```python
from build123d import *

# Parameters (mm, degrees)
EXTRUDE_THIN1_DEPTH = 372
SKETCH2_R           = 4.5
CUT_EXTRUDE1_DEPTH  = 447.144595395
LPATTERN1_COUNT     = 2
LPATTERN1_PITCH     = 320


with BuildPart() as part:
    # Sketch1 → Extrude-Thin1 (new body)
    with BuildSketch(Plane.XY):
        with BuildLine():
            Line((50, 206), (10, 206))
            ThreePointArc((10, 206), (2.928932188, 203.071067812), (0, 196))
            Line((0, 196), (0, 10))
            ThreePointArc((0, 10), (2.928932188, 2.928932188), (10, 0))
            Line((10, 0), (135, 0))
            Line((135, 0), (135, 5))
            Line((135, 5), (10, 5))
            ThreePointArc((10, 5), (6.464466094, 6.464466094), (5, 10))
            Line((5, 10), (5, 196))
            ThreePointArc((5, 196), (6.464466094, 199.535533906), (10, 201))
            Line((10, 201), (50, 201))
            Line((50, 201), (50, 206))
        make_face()
    extrude(amount=EXTRUDE_THIN1_DEPTH)

    # Sketch2 → Cut-Extrude1 (cut, through all)
    with BuildSketch(Plane(origin=(0, 206, 0), x_dir=(1, 0, 0), z_dir=(0, 1, 0))):
        with Locations(Location((27.5, -346, 0), (0, 0, 270))):
            Circle(SKETCH2_R)
    cut_extrude1 = extrude(amount=-CUT_EXTRUDE1_DEPTH, mode=Mode.SUBTRACT)

    # LPattern1: Cut-Extrude1 ×2
    with Locations(*[(0, 0, -i * LPATTERN1_PITCH) for i in range(1, LPATTERN1_COUNT)]):
        add(cut_extrude1, mode=Mode.SUBTRACT)


solid = part.part
```
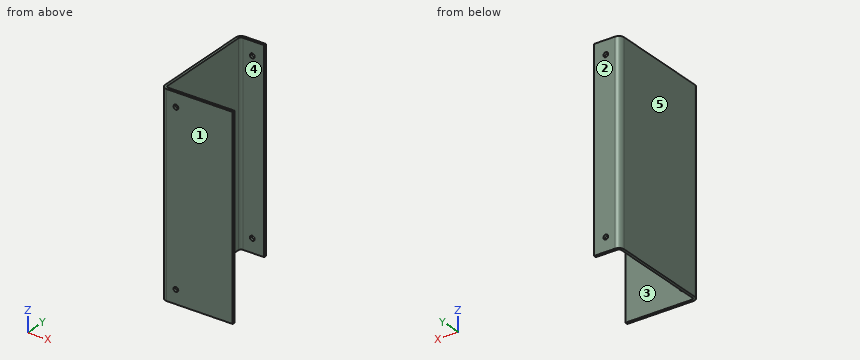
Geometry: final body of the model. Coordinates: model frame, mm. Face numbers are marked on the shaded views. A direction names the side the tool comes from. Coordinates: 2 decimals unless noted, no trailing zeros. Order: outer loops, then holes, each group sorted by start corner. A loop starts at its lowest first (then second) coordinate and runs counter-clockwise, first axis right, second up. Notation, with made-up numbers: (14, 65) - (47, 65) arc R21 cw to (47, 86) - close; hole circle Ø11 at (32.5, 53.5). An arc over 180 degrees is marked (long way). Return JSON: item names as keys, results as strings. Group by question number.
1. Cut plane A-A (x = 27.5). Output: boundary loops of the cut face in (y, z).
2. Material intervals for line 1 along Z through (x, y) = (27, 2); line 2 along Y through (x, z) = (45, 217.5); line 3 along X through (y, z) = (181.5, 139), sorted ascending. Write a range as [from, to].
3. Pull-direction query (Y, two-part tool) for the marked faces 1, 2 and 3; classes: pulls with the +Y half, pulls with the -Y half, needs draft (parallel to the pull), parting line crosses it, or undercut.
4. Pin query (flat end, axial travel): pin 1 (1 mm diameter, centred on x = 72.5, z = 85.5, fed in from +Y); pin 2 (7 mm diameter, centred on x = 27.5, z = 346, fed in from +Y); pin 3 (4 mm diameter, centred on y = 202.5, z = 272.5, fed in from +X). Return the tip coordinate at first contact, or that it passes through.
5. Cut plane D-D (x = 88). Output: boundary loops of the cut face in (y, z), plus the area to 3 significant figures.
6. Set-up query: the marked faces 4 and 5. Return all of +Z, -Z, +X, -X, +Y, -Y with unobstructed straight access to the full face (end or side cutting, diameter ignored); none if empty.
7. Cut plane C-C (z = 290). Output: boundary loops of the cut face in (x, y).
8. Cut plane B-B (z = 346). Output: boundary loops of the cut face in (x, y), plus the area to 3 significant figures.
Resolved:
{
 "1": {"outline": "(0, 0) - (5, 0) - (5, 21.5) - (0, 21.5) - close; (0, 30.5) - (5, 30.5) - (5, 341.5) - (0, 341.5) - close; (0, 350.5) - (5, 350.5) - (5, 372) - (0, 372) - close; (201, 0) - (206, 0) - (206, 21.5) - (201, 21.5) - close; (201, 30.5) - (206, 30.5) - (206, 341.5) - (201, 341.5) - close; (201, 350.5) - (206, 350.5) - (206, 372) - (201, 372) - close"},
 "2": {"line 1": "z = [0, 21.53], [30.47, 341.53], [350.47, 372]", "line 2": "y = [0, 5], [201, 206]", "line 3": "x = [0, 5]"},
 "3": {"face 1": "pulls with the -Y half", "face 2": "pulls with the +Y half", "face 3": "undercut"},
 "4": {"pin 1": "stops at y = 5", "pin 2": "passes through", "pin 3": "stops at x = 50"},
 "5": {"outline": "(0, 0) - (5, 0) - (5, 372) - (0, 372) - close", "area": "1,860 mm²"},
 "6": {"face 4": "+Z, -Z, +X", "face 5": "+Z, -Z, -X, +Y, -Y"},
 "7": {"outline": "(0, 10) arc R10 ccw to (10, 0) - (135, 0) - (135, 5) - (10, 5) arc R5 cw to (5, 10) - (5, 196) arc R5 cw to (10, 201) - (50, 201) - (50, 206) - (10, 206) arc R10 ccw to (0, 196) - close"},
 "8": {"outline": "(0, 10) arc R10 ccw to (10, 0) - (23, 0) - (23, 5) - (10, 5) arc R5 cw to (5, 10) - (5, 196) arc R5 cw to (10, 201) - (23, 201) - (23, 206) - (10, 206) arc R10 ccw to (0, 196) - close; (32, 0) - (135, 0) - (135, 5) - (32, 5) - close; (32, 201) - (50, 201) - (50, 206) - (32, 206) - close", "area": "1,780 mm²"}
}
